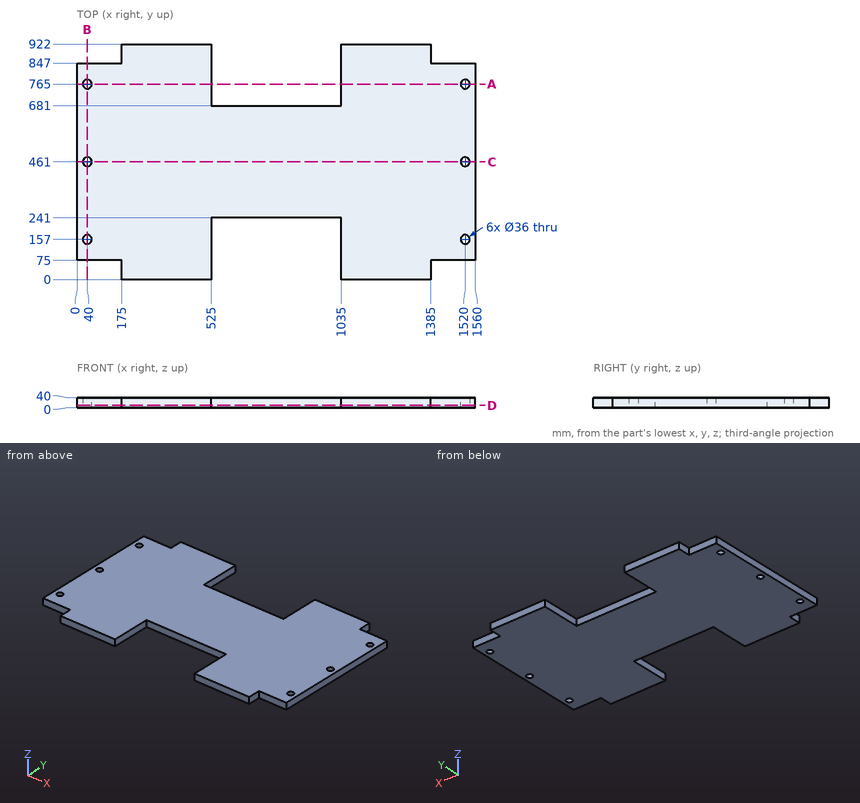
Answer from the drawing. Dimensions are ordinates in mm from the lowest x, y and z of the part. Give positions to 0.01 mm unless a question says otherwise; leave off trailing zeros. Order: outer loops, then holes, each group sorted by start corner. A loop starts at its lowest first (then second) coordinate and runs counter-clockwise, first axis right, second up. Notation, with made-up numbers: (70, 46) -> (100, 46) arc R16 cw to (100, 66) -> close; hole circle Ø1 at (-19, 51.5). An arc over 180 degrees is marked (long way). Answer as a JSON object with one key per item and string values. Group by question number.
1. Consider line 1 along Y through (x, z) = (1520, 21); line 2 along X through (y, z) = (765, 13); line 3 along X through (y, z) = (770.5, 12.5). Determine where each line is inside the solid, lowest interval first. Write a range as [from, to].
2. Section A-A on y = 765 is taken. Determine the outline of the cut face in (x, z).
3. Section D-D on z = 9.5 is taken. Determine the outline of the cut face in (x, y).
4. Section B-B on x = 40 is taken. Determine the outline of the cut face in (y, z).
5. Flat-ended cylindrical pins translate along their axes: pin 1 Ø20 at (x, z) = (871.5, 19) entering from +Y; pin 2 Ø12 at (x, z) = (128.5, 19) entering from -Y; pin 3 Ø20 at (y, z) = (33, 21.5) entering from -X; pin 4 Ø2 at (y, z) = (725, 24) entering from -X. Find the tip coordinate at first contact, or state that the pin passes through.
6. Section C-C on y = 461 is taken. Determine the outline of the cut face in (x, z).
Result sheet:
{
 "1": {"line 1": "y = [75, 139], [175, 443], [479, 747], [783, 847]", "line 2": "x = [0, 22], [58, 525], [1035, 1502], [1538, 1560]", "line 3": "x = [0, 22.86], [57.14, 525], [1035, 1502.86], [1537.14, 1560]"},
 "2": {"outline": "(0, 0) -> (22, 0) -> (22, 40) -> (0, 40) -> close; (58, 0) -> (525, 0) -> (525, 40) -> (58, 40) -> close; (1035, 0) -> (1502, 0) -> (1502, 40) -> (1035, 40) -> close; (1538, 0) -> (1560, 0) -> (1560, 40) -> (1538, 40) -> close"},
 "3": {"outline": "(0, 75) -> (175, 75) -> (175, 0) -> (525, 0) -> (525, 241) -> (1035, 241) -> (1035, 0) -> (1385, 0) -> (1385, 75) -> (1560, 75) -> (1560, 847) -> (1385, 847) -> (1385, 922) -> (1035, 922) -> (1035, 681) -> (525, 681) -> (525, 922) -> (175, 922) -> (175, 847) -> (0, 847) -> close; hole circle Ø36 at (40, 157); hole circle Ø36 at (40, 461); hole circle Ø36 at (40, 765); hole circle Ø36 at (1520, 157); hole circle Ø36 at (1520, 461); hole circle Ø36 at (1520, 765)"},
 "4": {"outline": "(75, 0) -> (139, 0) -> (139, 40) -> (75, 40) -> close; (175, 0) -> (443, 0) -> (443, 40) -> (175, 40) -> close; (479, 0) -> (747, 0) -> (747, 40) -> (479, 40) -> close; (783, 0) -> (847, 0) -> (847, 40) -> (783, 40) -> close"},
 "5": {"pin 1": "stops at y = 681", "pin 2": "stops at y = 75", "pin 3": "stops at x = 175", "pin 4": "stops at x = 0"},
 "6": {"outline": "(0, 0) -> (22, 0) -> (22, 40) -> (0, 40) -> close; (58, 0) -> (1502, 0) -> (1502, 40) -> (58, 40) -> close; (1538, 0) -> (1560, 0) -> (1560, 40) -> (1538, 40) -> close"}
}
